from build123d import *

# Parameters (mm, degrees)
BOSS_EXTRUDE_1_DEPTH = 645


with BuildPart() as part:
    # Sketch 1 → Boss-Extrude 1 (new, symmetric)
    with BuildSketch(Plane.XY):
        with BuildLine():
            Line((0, 50), (-40, 50))
            ThreePointArc((-40, 50), (-47.071067812, 47.071067812), (-50, 40))
            Line((-50, 40), (-50, 0))
            Line((-50, 0), (-50, -40))
            ThreePointArc((-50, -40), (-47.071067812, -47.071067812), (-40, -50))
            Line((-40, -50), (40, -50))
            ThreePointArc((40, -50), (47.071067812, -47.071067812), (50, -40))
            Line((50, -40), (50, 0))
            Line((50, 0), (50, 40))
            ThreePointArc((50, 40), (47.071067812, 47.071067812), (40, 50))
            Line((40, 50), (0, 50))
        make_face()
        with BuildLine():
            Line((0, 45), (-40, 45))
            ThreePointArc((-40, 45), (-43.535533906, 43.535533906), (-45, 40))
            Line((-45, 40), (-45, 0))
            Line((-45, 0), (-45, -40))
            ThreePointArc((-45, -40), (-43.535533906, -43.535533906), (-40, -45))
            Line((-40, -45), (40, -45))
            ThreePointArc((40, -45), (43.535533906, -43.535533906), (45, -40))
            Line((45, -40), (45, 0))
            Line((45, 0), (45, 40))
            ThreePointArc((45, 40), (43.535533906, 43.535533906), (40, 45))
            Line((40, 45), (0, 45))
        make_face(mode=Mode.SUBTRACT)
    extrude(amount=BOSS_EXTRUDE_1_DEPTH, both=True)


solid = part.part
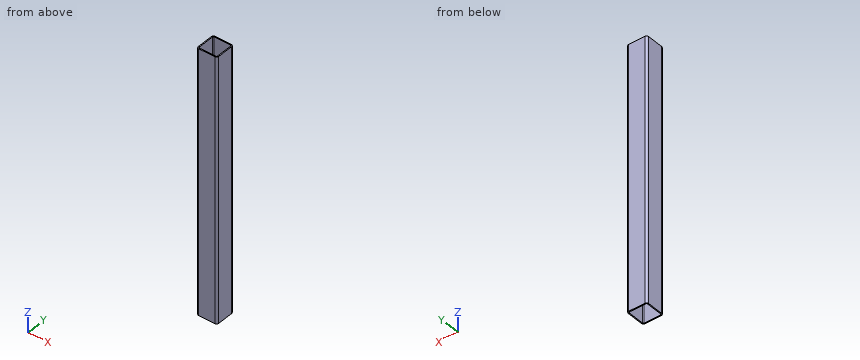
Check sheet for the modelled part. Datum: model origin and axes. Units: mm. Round coordinates to 2 decimals unless told otherwise and drop trailing zeros. Loops run counter-clockwise (first coordinate to the right, second up) from the corner with the lowest first, then second, coordinate; pieces in that order, holes last.
1. Sectioned sample at B-B on y = -24.5. Record the boundary of the cut face in (x, z), and give its area (3 significant figures).
2. Scan lines: probe 1 along Y at (x, z) = (40, 586.5); probe 2 along Y at (x, z) = (44.5, -197). Record each from-to range of solid material in increasing order.
3. Sectioned sample at A-A on z = 44. Record the boundary of the cut face in (x, y), and give its area (3 significant figures).
Recorded:
1. outline: (-50, -645) - (-45, -645) - (-45, 645) - (-50, 645) - close; (45, -645) - (50, -645) - (50, 645) - (45, 645) - close
1. area: 12,900 mm2
2. probe 1: y = -50 to -45, 45 to 50
2. probe 2: y = -48.93 to -42.18, 42.18 to 48.93
3. outline: (-50, -40) arc R10 ccw to (-40, -50) - (40, -50) arc R10 ccw to (50, -40) - (50, 40) arc R10 ccw to (40, 50) - (-40, 50) arc R10 ccw to (-50, 40) - close; hole (-45, -40) arc R5 ccw to (-40, -45) - (40, -45) arc R5 ccw to (45, -40) - (45, 40) arc R5 ccw to (40, 45) - (-40, 45) arc R5 ccw to (-45, 40) - close
3. area: 1,840 mm2
